Geometry: final body of the model. Coordinates: model frame, mm. A direction names the side the tool comes from. Coordinates: 2 decimals unless noted, no trailing zeros. Loops run counter-clockwise (first coordinate to the right, second up) from the corner with the lowest first, then second, coordinate; pieces in that order, holes last. Notation, with made-up numbers: (47.25, -24) - (81.25, -24) arc R6 ccw to (81.25, -13) - close; hole circle Ø1 at (21.5, 39). An arc over 180 degrees is marked (long way). Put each result on its own line as item: value. Start each with the question number.
1) Section D-D on z = 11.25. Output: boundary loops of the cut face in (x, y), and give its area (3 significant figures).
2) Section B-B on y = 0. Output: boundary loops of the cut face in (x, z), and give its area (3 significant figures).
3) Draft query along X for faces 1 (the flat face through (0, -5, 19)), 2 (the cylindrical face through (-0.055, -7.579, 9.213)), 3 (the cylindrical face through (-11, 0, 12)). Return one class per face: +X half, -X half, draft (parallel to the pull), parting line (faces both ways), or undercut.
4) Section A-A on x = 0. Output: boundary loops of the cut face in (y, z), and give its area (3 significant figures).
5) Material intervals for line 1 along Y through (x, z) = (0, 11.25); line 2 along Y through (x, z) = (3, 13), sorted ascending. Write a range as from..to.
6) Section C-C on z = 3. Output: boundary loops of the cut face in (x, y).
7) Contact query for flat-ended pins moving along their axis: pin 1 Ø5 at (x, y) = (-2, -4) entering from -Z; pin 2 Ø1.5 at (y, z) = (1.5, 2) entering from -X; pin 3 Ø12 at (x, y) = (3.5, -0.5) entering from -Z. Output: stop coordinate, or through.
8) Reachability of faces 4 (the flat face through (-6.491, 0.146, 4.794)), 5 (the cylindrical face through (-4.054, 1.277, 12.933)) from +Z, -Z, +X, -X, +Y, -Y: full face, straight path, thin tool, end or side. Return the list, or none.
```python
from build123d import *

# Parameters (mm, degrees)
SKETCH1_R              = 11
BOSS_EXTRUDE1_DEPTH    = 19
M10_TAPPED_HOLE1_D     = 8.5
M10_TAPPED_HOLE1_DEPTH = 24.5
M10_TAPPED_HOLE1_TIP   = 2.553657631
CUT_EXTRUDE1_DEPTH     = 12.5


with BuildPart() as part:
    # Sketch1 → Boss-Extrude1 (new body)
    with BuildSketch(Plane.XY):
        Circle(SKETCH1_R)
    extrude(amount=BOSS_EXTRUDE1_DEPTH)

    # M10 Tapped Hole1
    with Locations(Plane.XY.offset(19)):
        with Locations((0, 0)):
            Hole(M10_TAPPED_HOLE1_D / 2, depth=M10_TAPPED_HOLE1_DEPTH)
            with Locations((0, 0, -(M10_TAPPED_HOLE1_DEPTH + M10_TAPPED_HOLE1_TIP / 2))):  # 118° drill point
                Cone(0, M10_TAPPED_HOLE1_D / 2, M10_TAPPED_HOLE1_TIP, mode=Mode.SUBTRACT)

    # Sketch4 → Cut-Extrude1 (cut, symmetric)
    with BuildSketch(Plane(origin=(0, 0, 0), x_dir=(1, 0, 0), z_dir=(0, 1, 0))):
        with BuildLine():
            Line((3.535533906, -7.748737342), (28.284271247, 17))
            Line((28.284271247, 17), (0, 45.284271247))
            Line((0, 45.284271247), (-28.284271247, 17))
            Line((-28.284271247, 17), (-3.535533906, -7.748737342))
            ThreePointArc((-3.535533906, -7.748737342), (0, -9.213203436), (3.535533906, -7.748737342))
        make_face()
    extrude(amount=CUT_EXTRUDE1_DEPTH, both=True, mode=Mode.SUBTRACT)


solid = part.part
```
Answer block:
1. outline: circle Ø22 at (0, 0); hole circle Ø8.5 at (0, 0)
1. area: 323 mm²
2. outline: (-11, 0.28) - (-4.25, 7.03) - (-4.25, 19) - (-11, 19) - close; (4.25, 7.03) - (11, 0.28) - (11, 19) - (4.25, 19) - close
2. area: 207 mm²
3. face 1: draft
3. face 2: undercut
3. face 3: parting line
4. outline: (-11, 9.21) - (-4.25, 9.21) - (-4.25, 19) - (-11, 19) - close; (4.25, 9.21) - (11, 9.21) - (11, 19) - (4.25, 19) - close
4. area: 132 mm²
5. line 1: y = -11..-4.25, 4.25..11
5. line 2: y = -10.58..-3.01, 3.01..10.58
6. outline: (-8.28, -7.24) - (-8.28, 7.24) arc R11 ccw to start; (8.28, -7.24) arc R11 ccw to (8.28, 7.24) - close
7. pin 1: stops at z = 6.78
7. pin 2: stops at x = -10.97
7. pin 3: stops at z = 1.78
8. face 4: -Z, +Y, -Y
8. face 5: +Z, -Z
